```python
from build123d import *

# Parameters (mm, degrees)
EXTRUDE_1_DEPTH     = 740
SKETCH_2_W          = 53
SKETCH_2_H          = 5
CUT_EXTRUDE_1_DEPTH = 45
SKETCH_3_W          = 53
SKETCH_3_H          = 5
CUT_EXTRUDE_2_DEPTH = 45
SKETCH_4_W          = 53
SKETCH_4_H          = 5
CUT_EXTRUDE_3_DEPTH = 45


with BuildPart() as part:
    # 草图1 → 凸台-拉伸1 (new body)
    with BuildSketch(Plane.XY):
        Polygon((0, 0), (0, -120), (53, -120), (53, -115), (5, -115), (5, -5), (53, -5), (53, 0), align=None)
    extrude(amount=EXTRUDE_1_DEPTH)

    # 草图2 → 切除-拉伸1 (cut)
    with BuildSketch(Plane(origin=(0, 0, 0), x_dir=(-1, 0, 0), z_dir=(0, 0, -1))):
        with Locations((-26.5, -2.5)):
            Rectangle(SKETCH_2_W, SKETCH_2_H)
    extrude(amount=-CUT_EXTRUDE_1_DEPTH, mode=Mode.SUBTRACT)

    # 草图3 → 切除-拉伸2 (cut)
    with BuildSketch(Plane(origin=(0, 0, 0), x_dir=(-1, 0, 0), z_dir=(0, 0, -1))):
        with Locations((-26.5, -117.5)):
            Rectangle(SKETCH_3_W, SKETCH_3_H)
    extrude(amount=-CUT_EXTRUDE_2_DEPTH, mode=Mode.SUBTRACT)

    # 草图4 → 切除-拉伸3 (cut)
    with BuildSketch(Plane.XY.offset(740)):
        with Locations((26.5, -2.5)):
            Rectangle(SKETCH_4_W, SKETCH_4_H)
        with Locations((26.5, -117.5)):
            Rectangle(SKETCH_4_W, SKETCH_4_H)
    extrude(amount=-CUT_EXTRUDE_3_DEPTH, mode=Mode.SUBTRACT)


solid = part.part
```
CAD build for the part. Positions are in the model's coordinates, mm. A direction names the side the tool comes from. Round coordinates to 2 decimals unless told otherwise and drop trailing zeros. Order: outer loops, then holes, each group sorted by start corner. A loop starts at its lowest first (then second) coordinate and runs counter-clockwise, first axis right, second up. Notation, with made-up numbers: (-21, 44) -> (25, 44) arc R6 cw to (25, 50) -> close; hole circle Ø2 at (86, 43.5). An arc over 180 degrees is marked (long way). Write item = value, one per line.
(1) Cut at C-C (y = -16). Write the cut outline in (x, z), plus the area to 3 significant figures.
Answers follow:
outline = (0, 0) -> (5, 0) -> (5, 740) -> (0, 740) -> close
area = 3,700 mm²
(2) Flat gauge pins, fed straight in: P1, Ø2, axis at y = -20.5, z = 303, coming from the +X side; P2, Ø2.5, axis at x = 20.5, y = -117.5, coming from the -Z side; P3, Ø2.5, axis at x = 2.5, z = 22, coming from the +Y side. Where does each tip first touch, or does it go through?
Answers follow:
P1 = 5
P2 = 45
P3 = -5
(3) Cut at B-B (z = 478). Write the cut outline in (x, y), plus the area to 3 significant figures.
Answers follow:
outline = (0, -120) -> (53, -120) -> (53, -115) -> (5, -115) -> (5, -5) -> (53, -5) -> (53, 0) -> (0, 0) -> close
area = 1,080 mm²
(4) Cut at A-A (x = 44). Write the cut outline in (y, z).
Answers follow:
outline = (-120, 45) -> (-115, 45) -> (-115, 695) -> (-120, 695) -> close; (-5, 45) -> (0, 45) -> (0, 695) -> (-5, 695) -> close
(5) 3-axis set-ups, long thin cutter, end or side, ignore diameter. For faces 1 (the flat face through (0, -59, 365)), 2 (the flat face through (29, -115, 365)): which of +Z, -Z, +X, -X, +Y, -Y reach the whole face in a straight line?
Answers follow:
face_1 = +Z, -Z, -X, +Y, -Y
face_2 = +Z, -Z, +X
(6) Pull direction Y, two halves, no side cores. Call faces 3 (the flat face through (26, -120, 365)), 4 (the flat face through (5, -61, 365)), 5 (the flat face through (27, 0, 365)): +Y half, -Y half, draft (parallel to the pull), parting line (faces both ways), or undercut.
Answers follow:
face_3 = -Y half
face_4 = undercut
face_5 = +Y half
(7) Drill centre lines: L1, parallel to Y at x = 11, z = 582; L2, parallel to X at y = -43, z = 405. Where is each one in solid material? Low to high.
Answers follow:
L1 = -120 to -115, -5 to 0
L2 = 0 to 5
